Input: part model. Units: mm. Frame: model coordinates. A direction names the side the tool comes from. Round coordinates to 2 decimals unless told otherwise and drop trailing zeros. Order: outer loops, then holes, each group sorted by start corner. A loop starts at its lowest first (then second) coordinate and runs counter-clockwise, first axis right, second up.
Item 1: Cut plane A-A on y = 5.5. Output: boundary loops of the cut face in (x, z), then the cut area to 3 significant figures.
Item 2: Reachability of faces 1 (the flat face through (0.1, -22.3, 195)), 2 (the flat face through (-22, 0, 3)) from +Z, -Z, +X, -X, +Y, -Y: full face, straight path, thin tool, end or side. Return the list, or none.
Item 3: Line query: L1, parallel to X at y = -12.5, z = 25.5; L2, parallel to X at y = -21.5, z = 15. Output: solid intervals per line, ascending.
Item 4: Cut plane B-B on z = -53. Output: boundary loops of the cut face in (x, y), then the cut area to 3 significant figures.
Item 5: Mould query, pull axis Y, two halves, no side actions, for faces 3 (the flat face through (0, -25, 3)), 4 (the flat face through (0.1, -22.3, -195)), 5 (the flat face through (0, -22, 3)). Classes: released by +Y, released by -Y, zero draft, split by the parting line, or undercut.
```python
from build123d import *

# Parameters (mm, degrees)
GB_6728_1986_050_X_50_X_3_1_DEPTH = 390


with BuildPart() as part:
    # Sketch1 → Gb／6728-1986方形空心型钢 050 X 50 X 3(1) (new body)
    with BuildSketch(Plane.YX.offset(-195)):
        with BuildLine():
            Line((-19, -25), (19, -25))
            ThreePointArc((19, -25), (23.242640687, -23.242640687), (25, -19))
            Line((25, -19), (25, 19))
            ThreePointArc((25, 19), (23.242640687, 23.242640687), (19, 25))
            Line((19, 25), (-19, 25))
            ThreePointArc((-19, 25), (-23.242640687, 23.242640687), (-25, 19))
            Line((-25, 19), (-25, -19))
            ThreePointArc((-25, -19), (-23.242640687, -23.242640687), (-19, -25))
        make_face()
        with BuildLine():
            Line((-19, -22), (19, -22))
            ThreePointArc((19, -22), (21.121320344, -21.121320344), (22, -19))
            Line((22, -19), (22, 19))
            ThreePointArc((22, 19), (21.121320344, 21.121320344), (19, 22))
            Line((19, 22), (-19, 22))
            ThreePointArc((-19, 22), (-21.121320344, 21.121320344), (-22, 19))
            Line((-22, 19), (-22, -19))
            ThreePointArc((-22, -19), (-21.121320344, -21.121320344), (-19, -22))
        make_face(mode=Mode.SUBTRACT)
    extrude(amount=GB_6728_1986_050_X_50_X_3_1_DEPTH)


solid = part.part
```
From the geometry:
1. outline: (-25, -195) - (-22, -195) - (-22, 195) - (-25, 195) - close; (22, -195) - (25, -195) - (25, 195) - (22, 195) - close
1. area: 2,340 mm2
2. face 1: +Z, +X, -X, +Y, -Y
2. face 2: +Z, -Z
3. L1: x = -25 to -22, 22 to 25
3. L2: x = -24.45 to -20.66, 20.66 to 24.45
4. outline: (-25, -19) arc R6 ccw to (-19, -25) - (19, -25) arc R6 ccw to (25, -19) - (25, 19) arc R6 ccw to (19, 25) - (-19, 25) arc R6 ccw to (-25, 19) - close; hole (-22, -19) arc R3 ccw to (-19, -22) - (19, -22) arc R3 ccw to (22, -19) - (22, 19) arc R3 ccw to (19, 22) - (-19, 22) arc R3 ccw to (-22, 19) - close
4. area: 541 mm2
5. face 3: released by -Y
5. face 4: zero draft
5. face 5: undercut
